from build123d import *

# Parameters (mm, degrees)
HEX_BODY_6AF_X17_DEPTH        = 17
EDGE_CHAMFER_0_85_SIZE        = 0.85
HEX_TIP_PROFILE_4AF_OUTSIDE_W = 12.79
HEX_TIP_PROFILE_4AF_OUTSIDE_H = 11.862
HEX_TIP_4AF_X4_DEPTH          = 4


with BuildPart() as part:
    # Hex Body Profile 6AF → Hex Body 6AF x17 (new body)
    with BuildSketch(Plane(origin=(0, 0, 0), x_dir=(1, 0, 0), z_dir=(0, 1, 0))):
        Polygon((3.464101615, 0), (1.732050808, 3), (-1.732050808, 3), (-3.464101615, 0), (-1.732050808, -3), (1.732050808, -3), align=None)
    extrude(amount=HEX_BODY_6AF_X17_DEPTH)

    # Edge Chamfer 0.85
    edge_chamfer_0_85_edges = [part.edges().sort_by_distance(p)[0] for p in [
        (0, 0, 3),
        (-2.598076211, 0, 1.5),
        (-2.598076211, 0, -1.5),
        (0, 0, -3),
        (2.598076211, 0, -1.5),
        (2.598076211, 0, 1.5),
    ]]
    chamfer(edge_chamfer_0_85_edges, length=EDGE_CHAMFER_0_85_SIZE)

    # Hex Tip Profile 4AF outside → Hex Tip 4AF x4 (cut)
    with BuildSketch(Plane(origin=(0, 17, 0), x_dir=(1, 0, 0), z_dir=(0, 1, 0))):
        Rectangle(HEX_TIP_PROFILE_4AF_OUTSIDE_W, HEX_TIP_PROFILE_4AF_OUTSIDE_H)
        Polygon((2.309401077, 0), (1.154700538, 2), (-1.154700538, 2), (-2.309401077, 0), (-1.154700538, -2), (1.154700538, -2), align=None, mode=Mode.SUBTRACT)
    extrude(amount=-HEX_TIP_4AF_X4_DEPTH, mode=Mode.SUBTRACT)

    # Neck Groove Profile → Neck Groove (revolve, cut)
    with BuildSketch(Plane.XY):
        with BuildLine():
            Line((-3.464101615, 12.012038592), (-3.464101615, 13))
            Line((-3.464101615, 13), (-2.309401077, 13))
            ThreePointArc((-2.309401077, 13), (-2.659285909, 12.240164314), (-3.464101615, 12.012038592))
        make_face()
        with BuildLine():
            ThreePointArc((2.309401077, 12.012038592), (2.751182948, 10.926492222), (3.458298406, 9.991842624))
            Line((3.458298406, 9.991842624), (3.458298406, 12.012038592))
            Line((3.458298406, 12.012038592), (2.309401077, 12.012038592))
        make_face()
    revolve(axis=Axis((0, 17, 0), (0, -1, 0)), mode=Mode.SUBTRACT)

    # Hex Corner Turn Profile → Hex Corner Turn (revolve, cut)
    with BuildSketch(Plane.XY, mode=Mode.PRIVATE) as hex_corner_turn_sk:
        with BuildLine():
            Line((2.309401077, 16.837685955), (2.309401077, 13))
            Line((2.309401077, 13), (2.309401077, 12.012038592))
            ThreePointArc((2.309401077, 12.012038592), (2.751182948, 10.926492222), (3.458298406, 9.991842624))
            Line((3.458298406, 9.991842624), (11.092376237, 19.473540628))
            Line((11.092376237, 19.473540628), (2.309401077, 19.67629868))
            Line((2.309401077, 19.67629868), (2.309401077, 17))
            Line((2.309401077, 17), (2.309401077, 16.837685955))
        make_face()
    revolve(hex_corner_turn_sk.sketch.rotate(Axis((0, 0, 0), (0, 1, 0)), 179.8330498), axis=Axis((0, 0, 0), (0, 1, 0)), mode=Mode.SUBTRACT)

    # Tip Chamfer Profile → Tip Chamfer 0.5x45 (revolve, cut)
    with BuildSketch(Plane.XY, mode=Mode.PRIVATE) as tip_chamfer_0_5x45_sk:
        Polygon((-1.809401077, 17), (-2.309401077, 17), (-2.309401077, 16.5), align=None)
    revolve(tip_chamfer_0_5x45_sk.sketch.rotate(Axis((0, 17, 0), (0, -1, 0)), 90), axis=Axis((0, 17, 0), (0, -1, 0)), mode=Mode.SUBTRACT)


solid = part.part
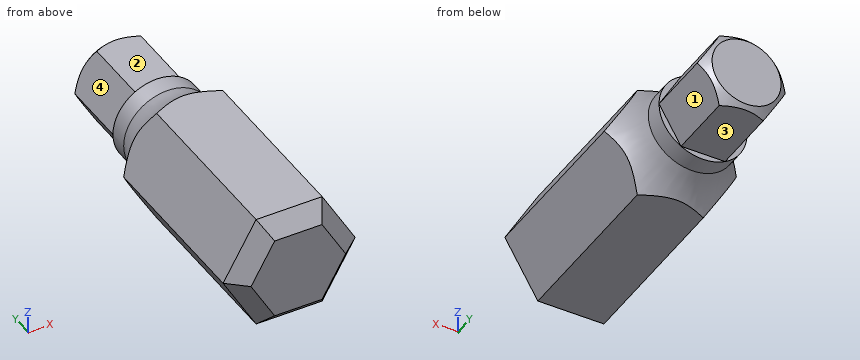
Work out the finished part from the listing and answer in its coordinate system (mm). Face numbers are marked on the shaded views. A direction names the side the tool comes from. Give positions to 0.01 mm unless a question says otherwise; leave off trailing zeros. Loops run counter-clockwise (first coordinate to the right, second up) from the corner with the lowest first, then second, coordinate; pieces in that order, holes last. Notation, with made-up numbers: (88.25, 26) -> (93.25, 26) arc R16 cw to (93.25, 44) -> close; hole circle Ø7 at (67.5, -8.75). An arc over 180 degrees is marked (long way). Use a Markdown table: item, result. Add a question column.
1. Section B-B on y = 2.5 is taken. Determine the outline of the cut face in (x, z), and give its area (3 significant figures).
2. Find the intervals of material crossed by probe 1 along Z at (x, y) = (-2.75, 2.75); probe 2 along X at (y, z) = (2.5, -1.5); probe 3 along X at (y, z) = (4.5, -0.5), in increasing order.
3. Section A-A on x = 0 is taken. Determine the outline of the cut face in (y, z).
4. For the marked faces 1, 2, 3 and 4, determine the directions among +Z, -Z, +X, -X, +Y, -Y from which every point of the face is accessible in a straight line to the end or side of a thin tool.
5. Flat-ended cylindrical pins translate along their axes: pin 1 Ø1.5 at (y, z) = (6, -2.5) entering from +X; pin 2 Ø2 at (x, z) = (3, 0.5) entering from +Y; pin 3 Ø1.5 at (y, z) = (7, -1.5) entering from +X. Find the tip coordinate at first contact, or state that the pin passes through.
6. Section C-C on y = 13.75 is taken. Determine the outline of the cut face in (x, z), and give its area (3 significant figures).
Results below:
| question | item | result |
|---|---|---|
| 1 | outline | (-3.46, 0) -> (-1.73, -3) -> (1.73, -3) -> (3.46, 0) -> (1.73, 3) -> (-1.73, 3) -> close |
| 1 | area | 31.2 mm^2 |
| 2 | probe 1 | z = -1.24 to 1.24 |
| 2 | probe 2 | x = -2.6 to 2.6 |
| 2 | probe 3 | x = -3.18 to 3.18 |
| 3 | outline | (0, -2.15) -> (0.85, -3) -> (10.54, -3) arc R4.5 cw to (12.01, -2.31) -> (13, -2.31) -> (13, -2) -> (16.81, -2) -> (17, -1.81) -> (17, 1.81) -> (16.81, 2) -> (13, 2) -> (13, 2.31) -> (12.01, 2.31) arc R4.5 cw to (10.54, 3) -> (0.85, 3) -> (0, 2.15) -> close |
| 4 | face 1 | -Z, +X, +Y |
| 4 | face 2 | +Z, +X, -X, +Y |
| 4 | face 3 | -Z, +X, -X, +Y |
| 4 | face 4 | +Z, -X, +Y |
| 5 | pin 1 | stops at x = 2.45 |
| 5 | pin 2 | stops at y = 16.77 |
| 5 | pin 3 | stops at x = 3.03 |
| 6 | outline | (-2.31, 0) -> (-1.15, -2) -> (1.15, -2) -> (2.31, 0) -> (1.15, 2) -> (-1.15, 2) -> close |
| 6 | area | 13.9 mm^2 |
